Build history of the part. All positions in model axes, mm. Face numbers are marked on the shaded views. Give positions to 0.01 mm unless a question says otherwise; leave off trailing zeros. Loops run counter-clockwise (first coordinate to the right, second up) from the corner with the lowest first, then second, coordinate; pieces in that order, holes last. Notation, with made-up numbers: (-3.75, 53.25) -> (14.25, 53.25) arc R17 ccw to (14.25, 67.25) -> close; hole circle Ø11 at (55, -33). An arc over 180 degrees is marked (long way). One line per question, with ' | ' between items. Start each with the question number.
(1) Drill centre lines: L1, parallel to Y at x = 2.5, z = 0 (3 decimals); L2, parallel to Z at x = 10.25, y = 2 (3 decimals); L3, parallel to Y at x = 6.25, z = 1.75 (3 decimals). Where is each one in solid material? Low to high. Write a range as from..to.
(2) Slice it at A-A, the plane x = 9.75. Write the cut outline in (y, z) (3 decimals), then the cut area to 3 significant figures.
(3) Mould opens along Z. For the marked faces 1, 2 and 3 say: pulls with the +Z half, pulls with the -Z half, needs draft (parallel to the pull), parting line crosses it, or undercut.
(4) Flat gauge pins, fed straight in: pin 1 Ø1.5 at (y, z) = (0, -1) entering from -X; pin 2 Ø1.5 at (x, y) = (13.5, -2.5) entering from +Z; pin 3 Ø3 at (y, z) = (-2, -2.5) entering from +X; pin 4 Ø2 at (y, z) = (-1, 1) entering from +X. Where does each tip first touch, or does it go through?
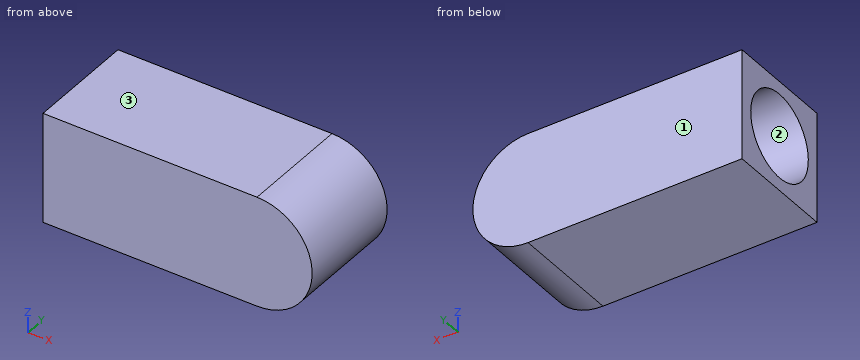
```python
from build123d import *

# Parameters (mm, degrees)
BOSS_EXTRUDE1_DEPTH = 3.175
SKETCH2_R           = 2.4384
CUT_EXTRUDE1_DEPTH  = 11.1125


with BuildPart() as part:
    # Sketch1 → Boss-Extrude1 (new, symmetric)
    with BuildSketch(Plane(origin=(0, 0, 0), x_dir=(1, 0, 0), z_dir=(0, 1, 0))):
        with BuildLine():
            Line((0, 3.175), (12.319, 3.175))
            ThreePointArc((12.319, 3.175), (15.494, 0), (12.319, -3.175))
            Line((12.319, -3.175), (0, -3.175))
            Line((0, -3.175), (0, 3.175))
        make_face()
    extrude(amount=BOSS_EXTRUDE1_DEPTH, both=True)

    # Sketch2 → Cut-Extrude1 (cut)
    with BuildSketch(Plane.ZY):
        Circle(SKETCH2_R)
    extrude(amount=-CUT_EXTRUDE1_DEPTH, mode=Mode.SUBTRACT)

    # Sketch3 → Cut-Revolve1 (revolve, cut)
    with BuildSketch(Plane(origin=(0, 0, 0), x_dir=(1, 0, 0), z_dir=(0, 1, 0))):
        Polygon((13.917558324, 0), (11.1125, -2.4384), (0, -2.4384), (0, 0), align=None)
    revolve(axis=Axis((0, 0, 0), (1, 0, 0)), mode=Mode.SUBTRACT)


solid = part.part
```
Final values:
1) L1: -3.175..-2.438, 2.438..3.175 | L2: -3.175..-1.395, 1.395..3.175 | L3: -3.175..-1.698, 1.698..3.175
2) outline: (-3.175, -3.175) -> (3.175, -3.175) -> (3.175, 3.175) -> (-3.175, 3.175) -> close; hole circle Ø4.877 at (0, 0) | area: 21.6 mm2
3) face 1: needs draft | face 2: undercut | face 3: pulls with the +Z half
4) pin 1: x = 11.9 | pin 2: z = 3.15 | pin 3: x = 15.33 | pin 4: x = 15.49
